from build123d import *

# Parameters (mm, degrees)
SKETCH_1_R           = 12.5
EXTRUDE_1_DEPTH      = 25
HOLE_WIZARD_M16_1_D  = 14
SKETCH_4_OUTSIDE_W   = 39.248
SKETCH_4_OUTSIDE_H   = 39.248
SKETCH_4_OUTSIDE_W_2 = 23
SKETCH_4_OUTSIDE_H_2 = 23
CUT_EXTRUDE_1_DEPTH  = 10
CHAMFER_1_SIZE       = 1


with BuildPart() as part:
    # 草图1 → 凸台-拉伸1 (new, symmetric)
    with BuildSketch(Plane(origin=(0, 0, 0), x_dir=(0, 0, -1), z_dir=(1, 0, 0))):
        Circle(SKETCH_1_R)
    extrude(amount=EXTRUDE_1_DEPTH, both=True)

    # M16 螺纹孔1 (through all)
    with Locations(Plane(origin=(25, 0, 0), x_dir=(0, 0, -1), z_dir=(1, 0, 0))):
        with Locations((0, 0)):
            Hole(HOLE_WIZARD_M16_1_D / 2)

    # 草图4 outside → 切除-拉伸1 (cut, symmetric)
    with BuildSketch(Plane(origin=(0, 0, 0), x_dir=(0, 0, -1), z_dir=(1, 0, 0))):
        Rectangle(SKETCH_4_OUTSIDE_W, SKETCH_4_OUTSIDE_H)
        Rectangle(SKETCH_4_OUTSIDE_W_2, SKETCH_4_OUTSIDE_H_2, mode=Mode.SUBTRACT)
    extrude(amount=CUT_EXTRUDE_1_DEPTH, both=True, mode=Mode.SUBTRACT)

    # 倒角1
    chamfer_1_edges = [part.edges().sort_by_distance(p)[0] for p in [
        (-25, 0, 12.5),
        (25, 0, 12.5),
        (25, 0, -7),
        (-25, 0, -7),
    ]]
    chamfer(chamfer_1_edges, length=CHAMFER_1_SIZE)


solid = part.part
Design review of the part built by this model. Coordinates are the model's own, in mm. A direction names the side the tool comes from. Coordinates: 2 decimals unless noted, no trailing zeros. Order: outer loops, then holes, each group sorted by start corner. A loop starts at its lowest first (then second) coordinate and runs counter-clockwise, first axis right, second up. Notation, with made-up numbers: (51, 64) -> (77, 64) arc R24 ccw to (77, 97) -> close; hole circle Ø4 at (3, -23.5). An arc over 180 degrees is marked (long way). Use one line per item in the form item = value. Start each with the question number.
(1) Add section C-C on x = -14. State the section outline as (y, z) points.
(2) Insertion check: pin 1 (3 mm diameter, centred on x = 11.5, z = -3, fed in from +Y); pin 2 (8 mm diameter, centred on x = -0.5, z = -4, fed in from -Y); pin 3 (0.8 mm diameter, centred on y = 12, z = -1.5, fed in from -X); pin 4 (10 mm diameter, centred on x = 7, z = -3.5, fed in from +Y). Each pin has a flat end and moves straight along its axis. Give the tip position at first contact, or say it passes through.
(3) Add section A-A on y = 0. State the section outline as (x, z) points.
(4) The part is to be moulded in two halves that separate along Y. For faces 5 (the cylindrical face through (0.34, 8.45, 9.21)), 6 (the flat face through (0, 0, -11.5)), 7 (the cylindrical face through (-0.336, -2.681, 6.466)), say which applies: +Y half, -Y half, draft (parallel to the pull), parting line (faces both ways), or undercut.
(5) For faces 1 (the flat face through (-10, 0, 12)), 2 (the flat face through (-10, -12, 0)), 3 (the flat face through (-10, 0, -12)), 4 (the flat face through (10, 12, 0)), list the 3-axis set-ups (+Z, -Z, +X, -X, +Y, -Y) from which the entire face can be reached by the end or side of a thin tool; tool diameter is ignored.
(6) For probe 1 along Y at (x, z) = (2.5, 0); probe 2 along Z at (x, y) = (18, 4.75); probe 3 along Z at (x, y) = (5.5, 4), list the stretches that pass through material, from the lowest coordinate up.
Answer block:
q1.outline = circle Ø25 at (0, 0); hole circle Ø14 at (0, 0)
q2.pin_1 = 12.41
q2.pin_2 = -11.5
q2.pin_3 = -24.81
q2.pin_4 = 12.5
q3.outline = (-25, -11.5) -> (-24, -12.5) -> (-10, -12.5) -> (-10, -11.5) -> (10, -11.5) -> (10, -12.5) -> (24, -12.5) -> (25, -11.5) -> (25, -8) -> (24, -7) -> (-24, -7) -> (-25, -8) -> close; (-25, 8) -> (-24, 7) -> (24, 7) -> (25, 8) -> (25, 11.5) -> (24, 12.5) -> (10, 12.5) -> (10, 11.5) -> (-10, 11.5) -> (-10, 12.5) -> (-24, 12.5) -> (-25, 11.5) -> close
q4.face_5 = parting line
q4.face_6 = draft
q4.face_7 = undercut
q5.face_1 = +Z, +Y, -Y
q5.face_2 = +Z, -Z, -Y
q5.face_3 = -Z, +Y, -Y
q5.face_4 = +Z, -Z, +Y
q6.probe_1 = -11.5 to -7, 7 to 11.5
q6.probe_2 = -11.56 to -5.14, 5.14 to 11.56
q6.probe_3 = -11.5 to -5.74, 5.74 to 11.5
